Here's how the part is built. I have some questions about the finished solid (model axes, mm). A direction names the side the tool comes from. Round coordinates to 2 decimals unless told otherwise and drop trailing zeros. Order: outer loops, then holes, each group sorted by start corner. A loop starts at its lowest first (then second) coordinate and runs counter-clockwise, first axis right, second up. Notation, with made-up numbers: (-14.75, 7) -> (43.25, 7) arc R10 ccw to (43.25, 15) -> close; hole circle Ø6 at (59, -35.5). An arc over 180 degrees is marked (long way). One line per item, written item: value.
```python
from build123d import *

# Parameters (mm, degrees)
SKETCH1_W                                           = 150
SKETCH1_H                                           = 160
BOSS_EXTRUDE1_DEPTH                                 = 20
SKETCH2_R                                           = 26
CUT_EXTRUDE1_DEPTH                                  = 14
SKETCH3_R                                           = 20
CUT_EXTRUDE2_DEPTH                                  = 14
M6_TAPPED_HOLE1_D                                   = 5
SKETCH9_R                                           = 29
CUT_EXTRUDE4_DEPTH                                  = 9
FILLET1_R                                           = 20
SKETCH10_W                                          = 150
SKETCH10_H                                          = 20
CUT_EXTRUDE5_DEPTH                                  = 2
HOLE_SIZE_BY_SOCKET_HEAD_CAP_SCREW_TYPE_D           = 9
HOLE_SIZE_BY_SOCKET_HEAD_CAP_SCREW_TYPE_CBORE_D     = 15
HOLE_SIZE_BY_SOCKET_HEAD_CAP_SCREW_TYPE_CBORE_DEPTH = 9


with BuildPart() as part:
    # Sketch1 → Boss-Extrude1 (new body)
    with BuildSketch(Plane.XZ):
        with Locations((75, -80)):
            Rectangle(SKETCH1_W, SKETCH1_H)
    extrude(amount=BOSS_EXTRUDE1_DEPTH)

    # Sketch2 → Cut-Extrude1 (cut)
    with BuildSketch(Plane.XZ.offset(20)):
        with Locations(Location((75, -115, 0), (0, 0, 270))):
            Circle(SKETCH2_R)
    extrude(amount=-CUT_EXTRUDE1_DEPTH, mode=Mode.SUBTRACT)

    # Sketch3 → Cut-Extrude2 (cut)
    with BuildSketch(Plane.XZ.offset(6)):
        with Locations(Location((75, -115, 0), (0, 0, 270))):
            Circle(SKETCH3_R)
    extrude(amount=-CUT_EXTRUDE2_DEPTH, mode=Mode.SUBTRACT)

    # M6 Tapped Hole1 (through all)
    with Locations(Plane(origin=(0, -20, 0), x_dir=(-1, 0, 0), z_dir=(0, -1, 0))):
        with Locations((-99.748737342, 139.748737342), (-50.251262658, 139.748737342), (-50.251262658, 90.251262658), (-99.748737342, 90.251262658)):
            Hole(M6_TAPPED_HOLE1_D / 2)

    # Sketch9 → Cut-Extrude4 (cut)
    with BuildSketch(Plane.XZ.offset(20)):
        with Locations(Location((75, -115, 0), (0, 0, 270))):
            Circle(SKETCH9_R)
    extrude(amount=-CUT_EXTRUDE4_DEPTH, mode=Mode.SUBTRACT)

    # Fillet1
    fillet1_edges = [part.edges().sort_by_distance(p)[0] for p in [
        (0, -10, 0),
        (150, -10, 0),
        (150, -10, -160),
        (0, -10, -160),
    ]]
    fillet(fillet1_edges, radius=FILLET1_R)

    # Sketch10 → Cut-Extrude5 (cut)
    with BuildSketch(Plane(origin=(0, 0, 0), x_dir=(1, 0, 0), z_dir=(0, 1, 0))):
        with Locations((75, 60)):
            Rectangle(SKETCH10_W, SKETCH10_H)
    extrude(amount=-CUT_EXTRUDE5_DEPTH, mode=Mode.SUBTRACT)

    # Hole size (by socket head cap screw type)1 (through all)
    with Locations(Plane(origin=(0, -20, 0), x_dir=(-1, 0, 0), z_dir=(0, -1, 0))):
        with Locations((-125, 60), (-25, 60), (-75, 15)):
            CounterBoreHole(HOLE_SIZE_BY_SOCKET_HEAD_CAP_SCREW_TYPE_D / 2, HOLE_SIZE_BY_SOCKET_HEAD_CAP_SCREW_TYPE_CBORE_D / 2, HOLE_SIZE_BY_SOCKET_HEAD_CAP_SCREW_TYPE_CBORE_DEPTH)


solid = part.part
```
Q1. For P1, Ø12, axis at x = 125, z = -60, coming from the +Y side; P2, Ø14.5, axis at x = 125, z = -60, coming from the -Y side, each with a flat end and sliding along its axis, tell me the tip position at first contact or that it passes through.
Answers:
P1: y = -2
P2: y = -11
Q2. I want a section at C-C on x = 75. Write out the boundary of the cut face in (y, z).
Answers:
outline: (-20, -160) -> (0, -160) -> (0, -135) -> (-6, -135) -> (-6, -141) -> (-11, -141) -> (-11, -144) -> (-20, -144) -> close; (-20, -86) -> (-11, -86) -> (-11, -89) -> (-6, -89) -> (-6, -95) -> (0, -95) -> (0, -70) -> (-2, -70) -> (-2, -50) -> (0, -50) -> (0, -19.5) -> (-11, -19.5) -> (-11, -22.5) -> (-20, -22.5) -> close; (-20, -7.5) -> (-11, -7.5) -> (-11, -10.5) -> (0, -10.5) -> (0, 0) -> (-20, 0) -> close
Q3. Which directions (+Z, -Z, +X, -X, +Y, -Y) give clear straight access to the entire face, cutting with the end or side of a thin tool? Please do faces 1 (the face through (120, -11, -60)), 2 (the face through (74, -20, -79)).
Answers:
face 1: -Y
face 2: +Z, -Z, +X, -X, -Y
Q4. I want a section at D-D on z = -15. Write out the boundary of the cut face in (x, y).
Answers:
outline: (0.64, -20) -> (67.5, -20) -> (67.5, -11) -> (70.5, -11) -> (70.5, 0) -> (0.64, 0) -> close; (79.5, -11) -> (82.5, -11) -> (82.5, -20) -> (149.36, -20) -> (149.36, 0) -> (79.5, 0) -> close
Q5. I need wall thicknesses on line 1 along X through (y, z) = (-5.25, -60); line 2 along X through (y, z) = (-14.25, -60); line 3 along Z through (x, y) = (125, -15.5). Which ranges of each line are inside material? Lowest first, please.
Answers:
line 1: 0 to 20.5, 29.5 to 120.5, 129.5 to 150
line 2: 0 to 17.5, 32.5 to 117.5, 132.5 to 150
line 3: -160 to -67.5, -52.5 to 0
Q6. If we mould it in two halves opening along Z, with no side actions, what happens to faces 3 (the face through (5.703, -10.14, -153.986)), 4 (the face through (97.765, -9.86, -88.73)), 5 (the face through (0, -10, -81))? For each: pulls with the +Z half, pulls with the -Z half, needs draft (parallel to the pull), parting line crosses it, or undercut.
Answers:
face 3: pulls with the -Z half
face 4: undercut
face 5: needs draft
Q7. I want a section at A-A on z = -60. Write out the boundary of the cut face in (x, y), then the cut area to 3 significant figures.
Answers:
outline: (0, -20) -> (17.5, -20) -> (17.5, -11) -> (20.5, -11) -> (20.5, -2) -> (0, -2) -> close; (29.5, -11) -> (32.5, -11) -> (32.5, -20) -> (117.5, -20) -> (117.5, -11) -> (120.5, -11) -> (120.5, -2) -> (29.5, -2) -> close; (129.5, -11) -> (132.5, -11) -> (132.5, -20) -> (150, -20) -> (150, -2) -> (129.5, -2) -> close
area: 2,270 mm2
Q8. I want a section at B-B on x = 125. Write out the boundary of the cut face in (y, z).
Answers:
outline: (-20, -160) -> (0, -160) -> (0, -70) -> (-2, -70) -> (-2, -64.5) -> (-11, -64.5) -> (-11, -67.5) -> (-20, -67.5) -> close; (-20, -52.5) -> (-11, -52.5) -> (-11, -55.5) -> (-2, -55.5) -> (-2, -50) -> (0, -50) -> (0, 0) -> (-20, 0) -> close
